Part print with two shaded views. Sizes in mm from the minimum x, y, z corner. A direction names the side the tool comes from. Give positions to 0.01 mm unless a question says otherwise; leave off trailing zeros. Loops run counter-clockwise (first coordinate to the right, second up) from the corner with the lowest first, then second, coordinate; pieces in that order, holes last. Notation, with made-up numbers: (81, 80) -> (92, 80) arc R27 cw to (92, 107) -> close; hole circle Ø1 at (47.5, 44). An arc over 180 degrees is marked (long way). One line per question, with ' | ' between items. Start each with the question number.
(1) Mould opens along Z. For the marked faces 1, 2 and 3 say: pulls with the +Z half, pulls with the -Z half, needs draft (parallel to the pull), parting line crosses it, or undercut.
(2) Slice it at C-C, the plane y = 12.5. Write the cut outline in (x, z).
(3) Drill centre lines: L1, parallel to Z at x = 9, y = 8.5; L2, parallel to X at y = 13.75, z = 9. Where is each one in solid material? Low to high. Write a range as from..to.
(4) Slice it at A-A, the plane z = 9. Write the cut outline in (x, y), then the cut area to 3 significant figures.
(5) Slice it at B-B, the plane y = 15. Write the cut outline in (x, z).
(6) 3-axis set-ups, long thin cutter, end or side, ignore diameter. For the marked faces 4 and 5: which of +Z, -Z, +X, -X, +Y, -Y reach the whole face in a straight line?
(7) Flat gauge pins, fed straight in: pin 1 Ø4 at (x, y) = (4, 8.5) entering from -Z; pin 2 Ø1.5 at (y, z) = (10.5, 11) entering from +X; pin 3 Ø3 at (x, y) = (14, 7) entering from +Z. Where does each tip first touch, or does it go through?
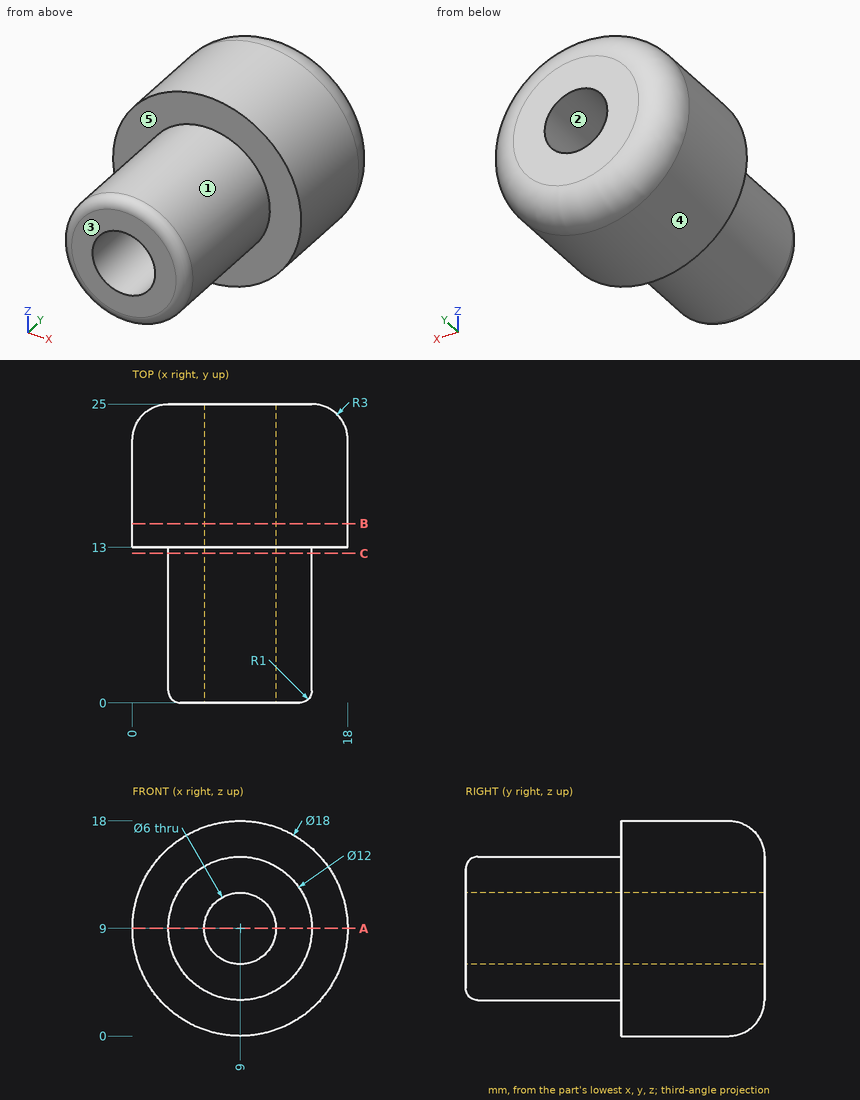
Final values:
1) face 1: parting line crosses it | face 2: undercut | face 3: needs draft
2) outline: circle Ø12 at (9, 9); hole circle Ø6 at (9, 9)
3) L1: 3..6, 12..15 | L2: 0..6, 12..18
4) outline: (0, 13) -> (3, 13) -> (3, 1) arc R1 ccw to (4, 0) -> (6, 0) -> (6, 25) -> (3, 25) arc R3 ccw to (0, 22) -> close; (12, 0) -> (14, 0) arc R1 ccw to (15, 1) -> (15, 13) -> (18, 13) -> (18, 22) arc R3 ccw to (15, 25) -> (12, 25) -> close | area: 218 mm2
5) outline: circle Ø18 at (9, 9); hole circle Ø6 at (9, 9)
6) face 4: +Y, -Y | face 5: -Y
7) pin 1: z = 3.8 | pin 2: x = 14.87 | pin 3: z = 13.87
